For this review, take the finished solid that the model builds, in its own axes (mm). Face numbers are marked on the shaded views. A direction names the side the tool comes from. Coordinates: 2 decimals unless noted, no trailing zeros. Order: outer loops, then holes, each group sorted by start corner. A loop starts at its lowest first (then second) coordinate and runs counter-clockwise, first axis right, second up.
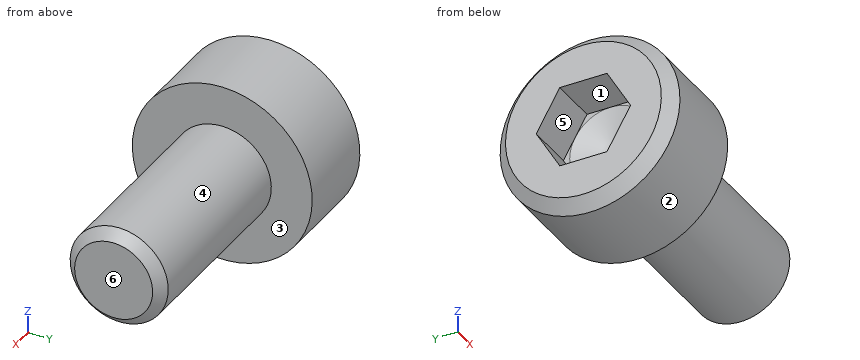
from build123d import *

# Parameters (mm, degrees)
CUT_EXTRUDE1_DEPTH = 1.5


with BuildPart() as part:
    # Sketch1 → Revolve1 (revolve)
    with BuildSketch(Plane.XY, mode=Mode.PRIVATE) as revolve1_sk:
        Polygon((-3, 0), (-3, 2.383333333), (-2.633333333, 2.75), (0, 2.75), (0, 1.5), (5.6928325, 1.5), (6, 1.1928325), (6, 0), align=None)
    revolve(revolve1_sk.sketch.rotate(Axis((6, 0, 0), (-1, 0, 0)), 270), axis=Axis((6, 0, 0), (-1, 0, 0)))

    # Sketch2 → Cut-Revolve1 (revolve, cut)
    with BuildSketch(Plane.XY, mode=Mode.PRIVATE) as cut_revolve1_sk:
        Polygon((-3, 0), (-3, 1.25), (-1.5, 1.25), (-1.165063509, 0), align=None)
    revolve(cut_revolve1_sk.sketch.rotate(Axis((-1.165063509, 0, 0), (-1, 0, 0)), 270), axis=Axis((-1.165063509, 0, 0), (-1, 0, 0)), mode=Mode.SUBTRACT)

    # Sketch3 → Cut-Extrude1 (cut)
    with BuildSketch(Plane(origin=(-3, 0, 0), x_dir=(0, 0, -1), z_dir=(1, 0, 0))):
        Polygon((-1.25, 0.721687836), (-1.25, -0.721687836), (0, -1.443375673), (1.25, -0.721687836), (1.25, 0.721687836), (0, 1.443375673), align=None)
    extrude(amount=CUT_EXTRUDE1_DEPTH, mode=Mode.SUBTRACT)


solid = part.part
1. To check wall thickness, follow L1, parallel to X at y = 0.6, z = 1.45; L2, parallel to Z at x = -0.5, y = -0.15; L3, parallel to Z at x = 3.5, y = 0.15. State the ranges of each line that lie inside material, in increasing order.
Answer below:
L1: x = -3 to 0
L2: z = -2.75 to 2.75
L3: z = -1.49 to 1.49
2. The part is to be moulded in two halves that separate along Z. For the marked faces 1, 2 and 3, say which applies: +Z half, -Z half, draft (parallel to the pull), parting line (faces both ways), or undercut.
Answer below:
face 1: undercut
face 2: parting line
face 3: draft
3. Clearance check with a flat-ended pin moving along its axis: pin 1 Ø1 at (x, y) = (-1.5, -2) entering from -Z. State where the tip first meets the part, or that it passes through.
Answer below:
pin 1: stops at z = -2.3
4. Machinability: for the marked faces 4, 5 and 6, which of the approach directions +Z, -Z, +X, -X, +Y, -Y give a long, thin tool a straight path to every point of the face, cutting with its end or side? Answer none if there is none.
Answer below:
face 4: +X
face 5: -X
face 6: +Z, -Z, +X, +Y, -Y
5. Take a section at B-B, the plane x = 1.5. Give the boundary of the cut face in (y, z), plus the area to 3 significant figures.
Answer below:
outline: circle Ø3 at (0, 0)
area: 7.07 mm2
6. Take a section at A-A, the plane x = -1. Give the boundary of the cut face in (y, z).
Answer below:
outline: circle Ø5.5 at (0, 0)
